```python
from build123d import *

# Parameters (mm, degrees)
EXTRUDE_1_DEPTH     = 329
SHELL_1_T           = -2
SKETCH_2_R          = 10
SKETCH_2_W          = 192
SKETCH_2_H          = 138
CUT_EXTRUDE_1_DEPTH = 658
SKETCH_3_W          = 30
SKETCH_3_H          = 658
EXTRUDE_2_DEPTH     = 2
EXTRUDE_3_DEPTH     = 2
SKETCH_5_R          = 4.5
CUT_EXTRUDE_2_DEPTH = 797
SKETCH_6_R          = 4.5
CUT_EXTRUDE_3_DEPTH = 10


with BuildPart() as part:
    # 草图1 → 凸台-拉伸1 (new, symmetric)
    with BuildSketch(Plane.XY):
        Polygon((0, 0), (-813, 0), (-813, 30), (-713.029639528, 100), (0, 100), align=None)
    extrude(amount=EXTRUDE_1_DEPTH, both=True)

    # 抽壳1
    shell_1_openings = [part.faces().sort_by_distance(p)[0] for p in [
        (-406.5, 0, 0),
    ]]
    offset(amount=SHELL_1_T, openings=shell_1_openings, kind=Kind.INTERSECTION)

    # 草图2 → 切除-拉伸1 (cut)
    with BuildSketch(Plane(origin=(0, 100, 0), x_dir=(1, 0, 0), z_dir=(0, 1, 0))):
        with Locations(Location((-613.029639528, 229, 0), (0, 0, 180))):
            Circle(SKETCH_2_R)
        with Locations(Location((-543.029639528, 229, 0), (0, 0, 180))):
            Circle(SKETCH_2_R)
        with Locations((-473.029639528, 229)):
            Circle(SKETCH_2_R)
        with Locations((-543.029639528, 80)):
            Rectangle(SKETCH_2_W, SKETCH_2_H)
    extrude(amount=-CUT_EXTRUDE_1_DEPTH, mode=Mode.SUBTRACT)

    # 草图3 → 凸台-拉伸2 (add)
    with BuildSketch(Plane.XZ):
        with Locations((13, 0)):
            Rectangle(SKETCH_3_W, SKETCH_3_H)
    extrude(amount=-EXTRUDE_2_DEPTH)

    # 草图4 → 凸台-拉伸3 (add)
    with BuildSketch(Plane.XZ):
        Polygon((-783, 299), (-783, -299), (0, -299), (0, -329), (-813, -329), (-813, 329), (0, 329), (0, 299), align=None)
    extrude(amount=-EXTRUDE_3_DEPTH)

    # 草图5 → 切除-拉伸2 (cut)
    with BuildSketch(Plane.XY.offset(329)):
        with Locations((-683.029639528, 84)):
            Circle(SKETCH_5_R)
        with Locations((-30, 84)):
            Circle(SKETCH_5_R)
    extrude(amount=-CUT_EXTRUDE_2_DEPTH, mode=Mode.SUBTRACT)

    # 草图6 → 切除-拉伸3 (cut)
    with BuildSketch(Plane.XZ):
        with Locations((-797, 299)):
            Circle(SKETCH_6_R)
        with Locations((-797, -299)):
            Circle(SKETCH_6_R)
        with Locations((-797, 0)):
            Circle(SKETCH_6_R)
    extrude(amount=-CUT_EXTRUDE_3_DEPTH, mode=Mode.SUBTRACT)


solid = part.part
```
The listing builds one solid part. Answer for the finished solid, in the listing's coordinates (mm). A direction names the side the tool comes from. Give positions to 0.01 mm unless a question says otherwise; leave off trailing zeros. Loops run counter-clockwise (first coordinate to the right, second up) from the corner with the lowest first, then second, coordinate; pieces in that order, holes last. Notation, with made-up numbers: M -8,-29.75 L 3,-29.75 A16 ccw 3,-16.75 Z; hole C 37.5,61.25 d4. An arc over 180 degrees is marked long. One line per item, written item: value.
Q1. Flat-ended cylindrical pins translate along their axes: P1, Ø5.5, axis at x = -797, z = 299, coming from the +Y side; P2, Ø2, axis at x = -58.5, z = 80, coming from the -Y side; P3, Ø1, axis at y = 99, z = -95, coming from the +X side. Find the tip coordinate at first contact, or state that the pin passes through.
Working result:
P1: stops at y = 43.13
P2: stops at y = 98
P3: stops at x = 0
Q2. Find the intervals of material crossed by line 1 (Z direction, x = -797, y = 0.6); line 2 (Z direction, x = -84.5, y = 81); line 3 (Y direction, x = -30, z = 328.05), in increasing order. Write a range as from..to.
Working result:
line 1: z = -329..-303.5, -294.5..-4.5, 4.5..294.5, 303.5..329
line 2: z = -329..-327, 327..329
line 3: y = 0..79.5, 88.5..100
Q3. A cutting plane is placed at B-B on z = -229. Determine the outline of the cut face in (x, y), then the cut area to 3 significant figures.
Working result:
outline: M -813,0 L -783,0 L -783,2 L -811,2 L -811,28.96 L -712.4,98 L -623.03,98 L -623.03,100 L -713.03,100 L -813,30 Z; M -603.03,98 L -553.03,98 L -553.03,100 L -603.03,100 Z; M -533.03,98 L -483.03,98 L -483.03,100 L -533.03,100 Z; M -463.03,98 L -2,98 L -2,0 L 28,0 L 28,2 L 0,2 L 0,100 L -463.03,100 Z
area: 1,910 mm^2
Q4. Determine the mould class of faces 4 (the face through (-533.04, 99.01, -228.56)), 5 (the face through (-387, 51, 329)), 6 (the face through (-391, 0, -315)), 7 (the face through (-387, 51, -329)) for opening direction Z: +Z half, -Z half, draft (parallel to the pull), parting line (faces both ways), or undercut.
Working result:
face 4: undercut
face 5: +Z half
face 6: draft
face 7: -Z half
Q5. A cutting plane is placed at D-D on x = -406. Determine the outline of the cut face in (y, z).
Working result:
outline: M 0,-329 L 100,-329 L 100,329 L 0,329 L 0,299 L 2,299 L 2,327 L 98,327 L 98,-327 L 2,-327 L 2,-299 L 0,-299 Z
Q6. For faces 1 (the face through (0, 52, 5)), 2 (the face through (-603.04, 99.01, -228.56)), 3 (the face through (-762.39, 62.996, 4.578)), determine the directions among +Z, -Z, +X, -X, +Y, -Y from which every point of the face is accessible in a straight line to the end or side of a thin tool.
Working result:
face 1: +Z, -Z, +X, +Y
face 2: +Y, -Y
face 3: none
Q7. A cutting plane is placed at A-A on z = -92. Determine the outline of the cut face in (x, y).
Working result:
outline: M -813,0 L -783,0 L -783,2 L -811,2 L -811,28.96 L -712.4,98 L -639.03,98 L -639.03,100 L -713.03,100 L -813,30 Z; M -447.03,98 L -2,98 L -2,0 L 28,0 L 28,2 L 0,2 L 0,100 L -447.03,100 Z
Q8. A cutting plane is placed at C-C on y = 67. Determine the outline of the cut face in (x, z).
Working result:
outline: M -760.16,-329 L 0,-329 L 0,329 L -760.16,329 Z; hole M -756.67,-327 L -2,-327 L -2,327 L -756.67,327 Z
